Build history of the part. All positions in model axes, mm. Face numbers are marked on the shaded views. A direction names the side the tool comes from. Round coordinates to 2 decimals unless told otherwise and drop trailing zeros. Write each loop counter-clockwise with the first axis right and the second up, starting at its lowest first coordinate (ties: lowest second). Pieces come first, ordered by that corner, then holes.
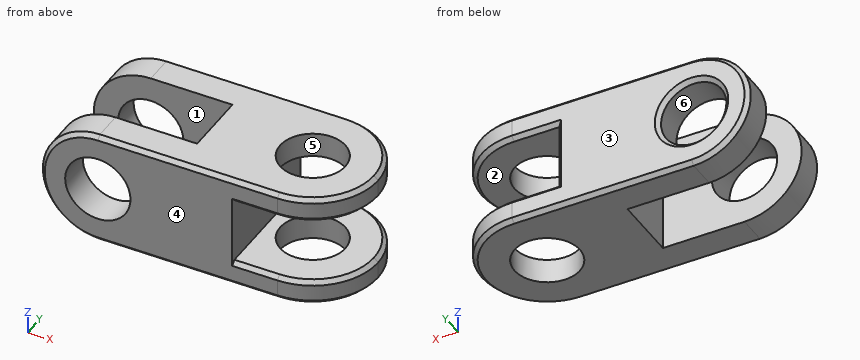
from build123d import *

# Parameters (mm, degrees)
SKETCH1_R               = 4
BOSS_EXTRUDE1_DEPTH     = 16
SKETCH2_W               = 13.535239133
SKETCH2_H               = 8
CUT_EXTRUDE1_DEPTH      = 16
SKETCH3_R               = 4
CUT_EXTRUDE2_DEPTH      = 16
CUT_EXTRUDE3_DEPTH      = 10
CUT_EXTRUDE3_DEPTH_BACK = 16
SKETCH4_W               = 14
SKETCH4_H               = 8
CHAMFER1_SIZE           = 0.5
SCALE1_SCALE            = 0.5


with BuildPart() as part:
    # Sketch1 → Boss-Extrude1 (new body)
    with BuildSketch(Plane(origin=(0, 0, 0), x_dir=(1, 0, 0), z_dir=(0, 1, 0))):
        with BuildLine():
            Line((0, 7), (30, 7))
            Line((30, 7), (30, -7))
            Line((30, -7), (0, -7))
            ThreePointArc((0, -7), (-7, 0), (0, 7))
        make_face()
        with Locations(Location((0, 0, 0), (0, 0, 270))):
            Circle(SKETCH1_R, mode=Mode.SUBTRACT)
    extrude(amount=BOSS_EXTRUDE1_DEPTH)

    # Sketch2 → Cut-Extrude1 (cut)
    with BuildSketch(Plane(origin=(0, 16, 0), x_dir=(1, 0, 0), z_dir=(0, 1, 0))):
        with Locations((23.232380434, 0)):
            Rectangle(SKETCH2_W, SKETCH2_H)
    extrude(amount=-CUT_EXTRUDE1_DEPTH, mode=Mode.SUBTRACT)

    # Sketch3 → Cut-Extrude2 (cut)
    with BuildSketch(Plane.XY.offset(7)):
        with BuildLine():
            Line((30, 16), (22, 16))
            ThreePointArc((22, 16), (27.656854238, 13.656854261), (30, 8.000000031))
            Line((30, 8.000000031), (30, 16))
        make_face()
        with BuildLine():
            Line((30, 0), (30, 8.000000031))
            ThreePointArc((30, 8.000000031), (27.656854261, 2.343145762), (22, 0))
            Line((22, 0), (30, 0))
        make_face()
        with Locations((22, 8)):
            Circle(SKETCH3_R)
    extrude(amount=-CUT_EXTRUDE2_DEPTH, mode=Mode.SUBTRACT)

    # Sketch4 → Cut-Extrude3 (cut, two sides: drawn at the far end of the back side and taken through both)
    with BuildSketch(Plane(origin=(0, 0, 0), x_dir=(0, 0, -1), z_dir=(1, 0, 0)).offset(-CUT_EXTRUDE3_DEPTH_BACK)):
        with Locations((0, 8)):
            Rectangle(SKETCH4_W, SKETCH4_H)
    extrude(amount=CUT_EXTRUDE3_DEPTH + CUT_EXTRUDE3_DEPTH_BACK, mode=Mode.SUBTRACT)

    # Chamfer1
    chamfer1_edges = [part.edges().sort_by_distance(p)[0] for p in [
        (0, 16, -4),
        (19.232380434, 0, 4),
        (16.464760867, 16, 0),
        (19.232380434, 16, 4),
        (19.232380434, 16, -4),
        (30, 8, -4),
        (11, 16, -7),
        (30, 8, 7),
        (-7, 16, 0),
        (30, 8, -7),
        (30, 8, 4),
        (11, 0, 7),
        (-7, 0, 0),
        (11, 0, -7),
        (19.232380434, 0, -4),
        (11, 16, 7),
    ]]
    chamfer(chamfer1_edges, length=CHAMFER1_SIZE)


with BuildPart() as part_1:
    # Scale1: scaled about (0, 0, 0)
    add(part.part.scale(SCALE1_SCALE))


solid = part_1.part
1) Slice it at A-A (z = 0). Write the cut outline in (x, y), plus the area to 3 significant figures.
Results:
outline: (-3.5, 0.25) - (-3.25, 0) - (-2, 0) - (-2, 2) - (-3.5, 2) - close; (-3.5, 6) - (-2, 6) - (-2, 7.75) - (-2.25, 8) - (-3.25, 8) - (-3.5, 7.75) - close; (2, 0) - (8.23, 0) - (8.23, 7.75) - (7.98, 8) - (2.25, 8) - (2, 7.75) - (2, 6) - (5, 6) - (5, 2) - (2, 2) - close
area: 43.7 mm2
2) Which spindle directions (+Z, -Z, +X, -X, +Y, -Y) get a long thin tool onto all of the face, cutting with end or side? Do the marked faces 1, 2 and 3. Say none if no direction does.
Results:
face 1: +Z, -Z, -X
face 2: +X, +Y, -Y
face 3: +Z, -Z, +X, -X, +Y
3) Mould opens along Y. For the marked faces 4, 5 and 6 say: released by +Y, released by -Y, zero draft, split by the parting line, or undercut.
Results:
face 4: released by -Y
face 5: undercut
face 6: zero draft
4) Slice it at B-B (x = 0.25). Count the separate pieces of the cut face and the enclosed holes in it, plus the area to 3 significant figures.
Results:
separate pieces: 4
enclosed holes: 0
area: 11.9 mm2
5) Wall check: L1, parallel to Z at x = 0, y = 6.8; L2, parallel to Y at x = 11, z = -2.9; L3, parallel to X at y = 7.1, z = 0. Give the ranges that are in metal, low to high.
Results:
L1: z = -3.5 to -2, 2 to 3.5
L2: y = 0 to 2, 6 to 8
L3: x = -3.5 to -2, 2 to 8.23
